Could you check a few things on this model? Use its own coordinates, in mm. A direction names the side the tool comes from. Give positions to 0.01 mm unless a question says otherwise; leave off trailing zeros.
from build123d import *

# Parameters (mm, degrees)
SKETCH_1_W                = 320
SKETCH_1_H                = 320
SKETCH_1_R                = 11.5
EXTRUDE_1_DEPTH           = 6
HOLE_WIZARD_M6_1_D        = 5
HOLE_WIZARD_1_D           = 9
HOLE_WIZARD_1_CBORE_D     = 15
HOLE_WIZARD_1_CBORE_DEPTH = 9
HOLE_WIZARD_M4_2_D        = 3.3
MIRROR_2_COPY_1_D         = 3.3
HOLE_WIZARD_M4_1_D        = 3.3
HOLE_WIZARD_M4_1_DEPTH    = 11.5
HOLE_WIZARD_M4_1_TIP      = 0.991420021


with BuildPart() as part:
    # 草图1 → 凸台-拉伸1 (new, symmetric)
    with BuildSketch(Plane.XY):
        Rectangle(SKETCH_1_W, SKETCH_1_H)
        with Locations((-130, 130)):
            Circle(SKETCH_1_R, mode=Mode.SUBTRACT)
        with Locations((130, 130)):
            Circle(SKETCH_1_R, mode=Mode.SUBTRACT)
        with Locations((130, -130)):
            Circle(SKETCH_1_R, mode=Mode.SUBTRACT)
        with Locations((-130, -130)):
            Circle(SKETCH_1_R, mode=Mode.SUBTRACT)
    extrude(amount=EXTRUDE_1_DEPTH, both=True)

    # M6 螺纹孔1 (through all)
    with Locations(Plane(origin=(0, 0, -6), x_dir=(-1, 0, 0), z_dir=(0, 0, -1))):
        with Locations((-36, 18), (-36, -18), (36, -18), (36, 18)):
            Hole(HOLE_WIZARD_M6_1_D / 2)

    # 打孔尺寸(%根据)内六角圆柱头螺钉的类型1 (through all)
    with Locations(Plane(origin=(0, 0, -6), x_dir=(-1, 0, 0), z_dir=(0, 0, -1))):
        with Locations((-45, 70), (45, 70), (45, -70), (-45, -70)):
            CounterBoreHole(HOLE_WIZARD_1_D / 2, HOLE_WIZARD_1_CBORE_D / 2, HOLE_WIZARD_1_CBORE_DEPTH)

    # M4 螺纹孔2 (through all)
    with Locations(Plane.XY.offset(6)):
        with Locations((-130, 146), (-114, 130), (-130, 114), (-146, 130)):
            hole_wizard_m4_2 = Hole(HOLE_WIZARD_M4_2_D / 2)

    # 镜向1: M4 螺纹孔2 across plane
    add(hole_wizard_m4_2.mirror(Plane.ZX), mode=Mode.SUBTRACT)

    # 镜向2: M4 螺纹孔2 across plane
    add(hole_wizard_m4_2.mirror(Plane(origin=(0, 0, 0), x_dir=(0, 0, 1), z_dir=(1, 0, 0))), mode=Mode.SUBTRACT)

    # 镜向2 copy 1 (through all)
    with Locations(Plane(origin=(0, 0, 6), x_dir=(-1, 0, 0), z_dir=(0, 0, 1))):
        with Locations((-130, 146), (-114, 130), (-130, 114), (-146, 130)):
            Hole(MIRROR_2_COPY_1_D / 2)

    # M4 螺纹孔1
    with Locations(Plane(origin=(0, 0, -6), x_dir=(-1, 0, 0), z_dir=(0, 0, -1))):
        with Locations((-7.5, 140), (7.5, 140)):
            Hole(HOLE_WIZARD_M4_1_D / 2, depth=HOLE_WIZARD_M4_1_DEPTH)
            with Locations((0, 0, -(HOLE_WIZARD_M4_1_DEPTH + HOLE_WIZARD_M4_1_TIP / 2))):  # 118° drill point
                Cone(0, HOLE_WIZARD_M4_1_D / 2, HOLE_WIZARD_M4_1_TIP, mode=Mode.SUBTRACT)


solid = part.part
Item 1: For faces 1 (the flat face through (160, -2, 0)), 2 (the cylindrical face through (41.539, 63.346, -1.563)), which set-ups out of +Z, -Z, +X, -X, +Y, -Y let a thin tool reach every point of the face, with its end or its side?
Findings:
face 1: +Z, -Z, +X, +Y, -Y
face 2: -Z
Item 2: Imagine slicing it at A-A on z = 1. Give the number of separate pieces and of enclosed holes in the cut face, then the cut area to 3 significant figures.
Findings:
separate pieces: 1
enclosed holes: 30
area: 99,800 mm2
Item 3: We'd pull the mould along Y, two halves only. Please class faces 3 (the flat face through (-50, 70, 3)), 4 (the flat face through (-2, 2, 6)), 5 (the flat face through (-2, 160, 0)): +Y half, -Y half, draft (parallel to the pull), parting line (faces both ways), or undercut.
Findings:
face 3: undercut
face 4: draft
face 5: +Y half
Item 4: Please list where these lines run through material, in increasing order: line 1 along Y through (x, z) = (-146, 2.5); line 2 along Y through (x, z) = (-36, 0); line 3 along Y through (x, z) = (7.5, 1.5).
Findings:
line 1: y = -160 to -131.65, -128.35 to 128.35, 131.65 to 160
line 2: y = -160 to -20.5, -15.5 to 15.5, 20.5 to 160
line 3: y = -160 to 138.35, 141.65 to 160
Item 5: For pin 1 (3 mm diameter, centred on x = 7.5, y = 140, fed in from -Z); pin 2 (7.5 mm diameter, centred on x = 43.5, y = -67.5, fed in from -Z); pin 3 (19.5 mm diameter, centred on x = 45, y = 70, fed in from +Z), each with a flat end and sliding along its axis, tell me the tip position at first contact or that it passes through.
Findings:
pin 1: stops at z = 5.59
pin 2: stops at z = 3
pin 3: stops at z = 6
